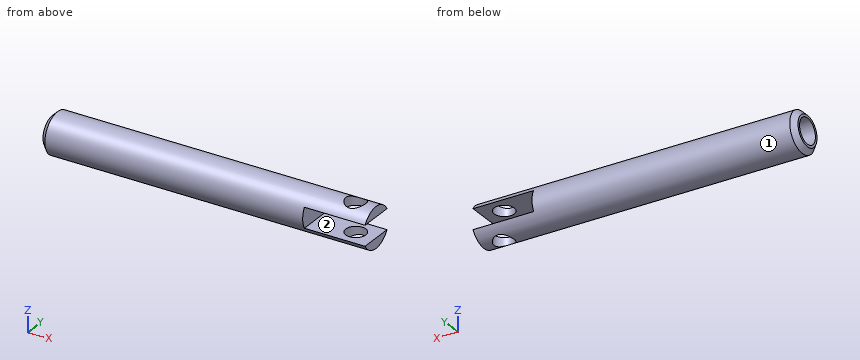
from build123d import *

# Parameters (mm, degrees)
ROD_PROFILE_SKETCH_W      = 4
ROD_PROFILE_SKETCH_H      = 0.25
END_NOTCH_SKETCH_R        = 0.125
END_NOTCH_CUT_DEPTH       = 5
CLEVIS_SLOT_SKETCH_W      = 0.75
CLEVIS_SLOT_SKETCH_H      = 0.25
CLEVIS_SLOT_DEPTH         = 5
CROSS_PIN_HOLE_SKETCH_R   = 0.15625
CROSS_PIN_HOLE_DEPTH      = 1.75
END_CHAMFER_SIZE          = 0.0625
SCALE_TO_FINAL_SIZE_SCALE = 25.4


with BuildPart() as part:
    # Rod Profile Sketch → Rod Body (revolve)
    with BuildSketch(Plane.XY, mode=Mode.PRIVATE) as rod_body_sk:
        with Locations((0, 0.125)):
            Rectangle(ROD_PROFILE_SKETCH_W, ROD_PROFILE_SKETCH_H)
    revolve(rod_body_sk.sketch.rotate(Axis((-2.293403827, 0, 0), (1, 0, 0)), 90), axis=Axis((-2.293403827, 0, 0), (1, 0, 0)))

    # End Notch Sketch → End Notch Cut (cut, symmetric)
    with BuildSketch(Plane.XY):
        with Locations((1.75, 0)):
            Circle(END_NOTCH_SKETCH_R)
    extrude(amount=END_NOTCH_CUT_DEPTH, both=True, mode=Mode.SUBTRACT)

    # Clevis Slot Sketch → Clevis Slot (cut, symmetric)
    with BuildSketch(Plane(origin=(0, 0, 0), x_dir=(1, 0, 0), z_dir=(0, 1, 0))):
        with Locations((1.625, 0)):
            Rectangle(CLEVIS_SLOT_SKETCH_W, CLEVIS_SLOT_SKETCH_H)
    extrude(amount=CLEVIS_SLOT_DEPTH, both=True, mode=Mode.SUBTRACT)

    # Cross Pin Hole Sketch → Cross Pin Hole (cut)
    with BuildSketch(Plane.ZY.offset(2)):
        Circle(CROSS_PIN_HOLE_SKETCH_R)
    extrude(amount=-CROSS_PIN_HOLE_DEPTH, mode=Mode.SUBTRACT)

    # End Chamfer
    end_chamfer_edges = [part.edges().sort_by_distance(p)[0] for p in [
        (-2, 0, -0.25),
    ]]
    chamfer(end_chamfer_edges, length=END_CHAMFER_SIZE)


with BuildPart() as part_1:
    # Scale to Final Size: scaled about (0, 0, 0)
    add(part.part.scale(SCALE_TO_FINAL_SIZE_SCALE))


solid = part_1.part
CAD build for the part. Positions are in the model's coordinates, mm. Face numbers are marked on the shaded views. Round coordinates to 2 decimals unless told otherwise and drop trailing zeros. Order: outer loops, then holes, each group sorted by start corner. A loop starts at its lowest first (then second) coordinate and runs counter-clockwise, first axis right, second up. Notation, with made-up numbers: (26, 57) - (52, 57) arc R18 cw to (52, 87) - close; hole circle Ø8 at (58.25, -35.75). An arc over 180 degrees is marked (long way). Return JSON: item names as keys, results as strings.
(1) Pull direction Z, two halves, no side cores. Call the marked faces 1 and 2: +Z half, -Z half, draft (parallel to the pull), parting line (faces both ways), or undercut.
Answer key:
{"face 1": "parting line", "face 2": "undercut"}
(2) Cut at D-D (y = 1.75). State how many separate pieces and enclosed holes the cut face has, then the cut area to 3 significant figures.
Answer key:
{"separate pieces": "3", "enclosed holes": "0", "area": "769 mm^2"}
(3) Pin check, flat tips, straight feed: pin 1 Ø2 at (x, y) = (8.5, -4.5) entering from +Z; pin 2 Ø1.5 at (x, y) = (-33, 1.5) entering from +Z; pin 3 Ø5.5 at (x, y) = (44.45, 0) entering from +Z; pin 4 Ø4 at (y, z) = (0, -1.5) entering from -X. Stop position of each tip, or through.
Answer key:
{"pin 1": "stops at z = 5.3", "pin 2": "stops at z = 6.31", "pin 3": "passes through", "pin 4": "stops at x = -6.35"}
(4) Wall check: probe 1 along Y at (x, z) = (-37, 0); probe 2 along Z at (x, y) = (40, 0.5) (3 decimals); probe 3 along X at (y, z) = (-1, -2.5). Give the ranges that are in metal, low to high. Write a range as from..to.
Answer key:
{"probe 1": "y = -6.35..-3.97, 3.97..6.35", "probe 2": "z = -6.33..-3.175, 3.175..6.33", "probe 3": "x = -6.35..31.75"}
(5) Cut at A-A (x = 44.45). Give the cut face in (y, z) (3 decimals), then the cut area to 3 significant figures.
Answer key:
{"outline": "(-5.499, -3.175) arc R6.35 ccw to (-3.175, -5.499) - (-3.175, -3.175) - close; (-5.499, 3.175) - (-3.175, 3.175) - (-3.175, 5.499) arc R6.35 ccw to start; (3.175, -5.499) arc R6.35 ccw to (5.499, -3.175) - (3.175, -3.175) - close; (3.175, 3.175) - (5.499, 3.175) arc R6.35 ccw to (3.175, 5.499) - close", "area": "12.7 mm^2"}
(6) Cut at B-B (z = 0). Give the cut face in (x, y).
Answer key:
{"outline": "(-50.8, -4.76) - (-49.21, -6.35) - (31.75, -6.35) - (31.75, 6.35) - (-49.21, 6.35) - (-50.8, 4.76) - (-50.8, 3.97) - (-6.35, 3.97) - (-6.35, -3.97) - (-50.8, -3.97) - close"}
(7) Cut at C-C (x = 13.5). Give the cut face in (y, z), then the cut area to 3 significant figures.
Answer key:
{"outline": "circle Ø12.7 at (0, 0)", "area": "127 mm^2"}
